Geometry: final body of the model. Coordinates: model frame, mm. Round coordinates to 2 decimals unless told otherwise and drop trailing zeros. Loops run counter-clockwise (first coordinate to the right, second up) from the corner with the lowest first, then second, coordinate; pieces in that order, holes last. Notation, with made-up numbers: (75.5, -13.75) -> (119.5, -13.75) arc R35 ccw to (119.5, 22.25) -> close; hole circle Ø3 at (67.5, 13.5). An arc over 180 degrees is marked (long way). Answer in a Markdown table with one row per item.
```python
from build123d import *

# Parameters (mm, degrees)
EXTRUDE_1_DEPTH        = 1100
SKETCH_2_R             = 2.5
CUT_EXTRUDE_1_DEPTH    = 1101.846946673
PATTERN_LINEAR_1_COUNT = 5
PATTERN_LINEAR_1_PITCH = 260


with BuildPart() as part:
    # 草图1 → 凸台-拉伸1 (new body)
    with BuildSketch(Plane.XY):
        Polygon((0, 0), (0, -10), (40, -10), (40, 0), (42, 0), (42, -12), (-2, -12), (-2, 0), align=None)
    extrude(amount=EXTRUDE_1_DEPTH)

    # 草图2 → 切除-拉伸1 (cut, through all)
    with BuildSketch(Plane(origin=(0, -10, 0), x_dir=(1, 0, 0), z_dir=(0, 1, 0))):
        with Locations(Location((20, -30, 0), (0, 0, 270))):
            Circle(SKETCH_2_R)
    cut_extrude_1 = extrude(amount=-CUT_EXTRUDE_1_DEPTH, mode=Mode.SUBTRACT)

    # 阵列(线性)1: 切除-拉伸1 ×5
    with Locations(*[(0, 0, i * PATTERN_LINEAR_1_PITCH) for i in range(1, PATTERN_LINEAR_1_COUNT)]):
        add(cut_extrude_1, mode=Mode.SUBTRACT)


solid = part.part
```
Item 1: Section query C-C, the plane x = 7.5. Output: boundary loops of the cut face in (y, z).
Ans:
| item | result |
|---|---|
| outline | (-12, 0) -> (-10, 0) -> (-10, 1100) -> (-12, 1100) -> close |
Item 2: Section query B-B, the plane z = 518.5. Output: boundary loops of the cut face in (x, y).
Ans:
| item | result |
|---|---|
| outline | (-2, -12) -> (42, -12) -> (42, 0) -> (40, 0) -> (40, -10) -> (0, -10) -> (0, 0) -> (-2, 0) -> close |
Item 3: Ray query, L1, parallel to Z at x = 21, y = -11; L2, parallel to X at y = -1, z = 365; L3, parallel to X at y = -10.9, z = 1070. Return the intervals inside material, ascending.
Ans:
| item | result |
|---|---|
| L1 | 0 to 27.71, 32.29 to 287.71, 292.29 to 547.71, 552.29 to 807.71, 812.29 to 1067.71, 1072.29 to 1100 |
| L2 | -2 to 0, 40 to 42 |
| L3 | -2 to 17.5, 22.5 to 42 |
Item 4: First-contact query: P1, Ø6.5, axis at x = 20, z = 550, coming from the +Y side. Flat tip, straight axial feed; report the tip coordinate or a pass-through.
Ans:
| item | result |
|---|---|
| P1 | y = -10 |
Item 5: Section query A-A, the plane y = -5.5. Output: boundary loops of the cut face in (x, z).
Ans:
| item | result |
|---|---|
| outline | (-2, 0) -> (0, 0) -> (0, 1100) -> (-2, 1100) -> close; (40, 0) -> (42, 0) -> (42, 1100) -> (40, 1100) -> close |
Item 6: Mould query, pull axis X, two halves, no side actions, for faces 1 (the flat face through (20, -10, 542)), 2 (the flat face through (20, -12, 542)). Classes: released by +X, released by -X, zero draft, split by the parting line, or undercut.
Ans:
| item | result |
|---|---|
| face 1 | undercut |
| face 2 | zero draft |
